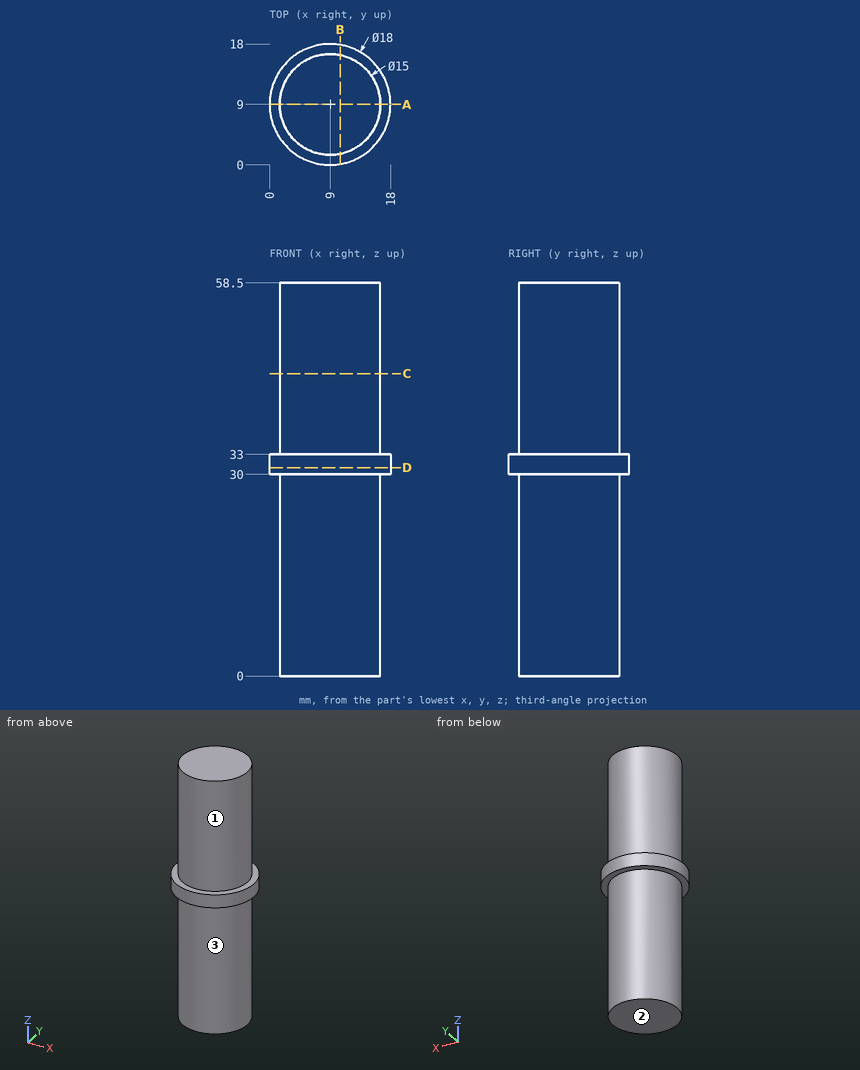
Study the drawing (mm; zero at the part's minimum x, y, z) and answer. A direction names the side the tool comes from. Coordinates: 2 decimals unless noted, no trailing zeros. Loops run counter-clockwise (first coordinate to the right, second up) from the corner with the lowest first, then second, coordinate; pieces in that order, holes last. Notation, with made-up numbers: (-11.5, -36) -> (18.5, -36) arc R16 cw to (18.5, -20) -> close; hole circle Ø8 at (78, 89.5). An arc over 180 degrees is marked (long way). Answer in a Markdown table with one row per item. Add a question column.
1. Consider line 1 (Z direction, x = 1.75, y = 4); line 2 (X direction, y = 9.25, z = 34); line 3 (X direction, y = 10, z = 19.5). Determine where each line is inside the solid, lowest interval first. Write a range as [from, to].
2. The part is cut by section D-D, the plane z = 31. Write down the section's boundary in (x, y).
3. Flat-ended cylindrical pins translate along their axes: P1, Ø4, axis at y = 8, z = 41, coming from the +X side; P2, Ø1.5, axis at x = 14, z = 6, coming from the -Y side; P3, Ø10, axis at x = 6.5, z = 52.5, coming from the -Y side. Find the tip coordinate at first contact, or state that the pin passes through.
4. For the marked faces 1, 2 and 3, determine the directions among +Z, -Z, +X, -X, +Y, -Y from which every point of the face is accessible in a straight line to the end or side of a thin tool.
5. The part is cut by section A-A, the plane y = 9. Write down the section's boundary in (x, z), then the cut area to 4 significant figures.
6. The part is cut by section B-B, the plane x = 10.5. Write down the section's boundary in (y, z), then the cut area to 3 significant figures.
7. The part is cut by section C-C, the plane z = 45. Write down the section's boundary in (x, y).
Answer below:
| question | item | result |
|---|---|---|
| 1 | line 1 | [30, 33] |
| 1 | line 2 | [1.5, 16.5] |
| 1 | line 3 | [1.57, 16.43] |
| 2 | outline | circle Ø18 at (9, 9) |
| 3 | P1 | x = 16.5 |
| 3 | P2 | y = 2.82 |
| 3 | P3 | y = 1.5 |
| 4 | face 1 | +Z |
| 4 | face 2 | -Z, +X, -X, +Y, -Y |
| 4 | face 3 | -Z |
| 5 | outline | (0, 30) -> (1.5, 30) -> (1.5, 0) -> (16.5, 0) -> (16.5, 30) -> (18, 30) -> (18, 33) -> (16.5, 33) -> (16.5, 58.5) -> (1.5, 58.5) -> (1.5, 33) -> (0, 33) -> close |
| 5 | area | 886.5 mm2 |
| 6 | outline | (0.13, 30) -> (1.65, 30) -> (1.65, 0) -> (16.35, 0) -> (16.35, 30) -> (17.87, 30) -> (17.87, 33) -> (16.35, 33) -> (16.35, 58.5) -> (1.65, 58.5) -> (1.65, 33) -> (0.13, 33) -> close |
| 6 | area | 869 mm2 |
| 7 | outline | circle Ø15 at (9, 9) |
